Model file for the job. Use its own axes, mm. A direction names the side the tool comes from. Coordinates: 2 decimals unless noted, no trailing zeros. Write each loop counter-clockwise with the first axis right and the second up, starting at its lowest first coordinate (ties: lowest second). Pieces come first, ordered by that corner, then holes.
Q1. Band-saw the part on C-C, the plane z = 75.5. Write the cut outline in (x, y).
Q2. Which spindle directions (+Z, -Z, +X, -X, +Y, -Y) get a long thin tool onto all of the face, cutting with end or side? Do faces 1 (the flat face through (-16, -60, 16)), 2 (the flat face through (-20, -65, 54)), 3 (the flat face through (-1, -22, 32)), 4 (the flat face through (-54, -51, 20)), 5 (the flat face through (38, -51, 47)). Say none if no direction does.
Q3. Pull direction Y, two halves, no side cores. Call faces 6 (the flat face through (-29.126, -44.386, 54.477)), 7 (the flat face through (16, -60, 16)), 8 (the cylindrical face through (28.874, -66.959, 79.932)): released by +Y, released by -Y, zero draft, split by the parting line, or undercut.
Q4. Band-saw the part on B-B, the plane y = -15.5. Write the cut outline in (x, z), plus the area to 3 significant figures.
Q5. Pin check, flat tips, straight feed: P1, Ø16, axis at x = -4.5, z = 17, coming from the -Y side; P2, Ø3, axis at x = 29.5, y = 25, coming from the +Z side; P3, Ø5, axis at y = -61.5, z = 57.5, coming from the +X side; P4, Ø14.5, axis at y = -68, z = 72, coming from the -X side. Stop position of each tip, or through.
Q6. Band-saw the part on D-D, the plane x = 54. Write the cut outline in (y, z), plus the area to 3 significant figures.
Q7. Band-saw the part on A-A, the plane x = 0. Write the cut outline in (y, z).
Q8. Drill centre lines: probe 1 along Y at (x, z) = (-54, 8.5); probe 2 along X at (y, z) = (-65, 56); probe 3 along X at (y, z) = (-35.5, 15.5). Where is each one in solid material? Low to high.
from build123d import *

# Parameters (mm, degrees)
BASE_BLOCK_DEPTH              = 32
FORK_ARMS_DEPTH               = 20
SIDE_FLANGE_DEPTH             = 18
FLANGE_START                  = -18
FLANGE_EXTENSION_DEPTH        = 18
FORK_SLOT_SKETCH_W            = 32
FORK_SLOT_SKETCH_H            = 48
FORK_SLOT_48X32_DEPTH         = 123.849501423
FORK_ARM_PROFILE_CUT_SKETCH_R = 8
FORK_ARM_PROFILE_CUT_DEPTH    = 129.763348823
FLANGE_HOLES_SKETCH_R         = 8
FLANGE_HOLES_16_DEPTH         = 163.677595261
PIVOT_BORE_SKETCH_R           = 20
PIVOT_BORE_40_DEPTH           = 123.849501423


with BuildPart() as part:
    # Base Block Sketch → Base Block (new body)
    with BuildSketch(Plane.XY):
        with BuildLine():
            Line((-38, 0), (-38, -84))
            Line((-38, -84), (38, -84))
            Line((38, -84), (38, 0))
            ThreePointArc((38, 0), (0, 38), (-38, 0))
        make_face()
    extrude(amount=BASE_BLOCK_DEPTH)

    # Fork Arms Sketch → Fork Arms (add)
    with BuildSketch(Plane(origin=(0, 0, 0), x_dir=(-1, 0, 0), z_dir=(0, 0, -1))):
        with BuildLine():
            Line((38, -84), (70, -84))
            Line((70, -84), (70, -27.712812921))
            ThreePointArc((70, -27.712812921), (47.66969722, -21.166010489), (38, 0))
            Line((38, 0), (38, -84))
        make_face()
        with BuildLine():
            Line((-38, -84), (-70, -84))
            Line((-70, -84), (-70, -27.712812921))
            ThreePointArc((-70, -27.712812921), (-47.66969722, -21.166010489), (-38, 0))
            Line((-38, 0), (-38, -84))
        make_face()
    extrude(amount=-FORK_ARMS_DEPTH)

    # Side Flange Sketch → Side Flange (add)
    with BuildSketch(Plane.ZY.offset(38)):
        with BuildLine():
            Line((72, -84), (32, -84))
            Line((32, -84), (32, -36))
            Line((32, -36), (77.592604925, -53.009243843))
            ThreePointArc((77.592604925, -53.009243843), (87.745667634, -70.841469822), (72, -84))
        make_face()
    extrude(amount=-SIDE_FLANGE_DEPTH)

    # Flange Extension Sketch → Flange Extension (add)
    with BuildSketch(Plane(origin=(38, 0, 0), x_dir=(0, 0, -1), z_dir=(1, 0, 0)).offset(FLANGE_START)):
        with BuildLine():
            Line((-72, -84), (-32, -84))
            Line((-32, -84), (-32, -36))
            Line((-32, -36), (-77.592604925, -53.009243843))
            ThreePointArc((-77.592604925, -53.009243843), (-87.745667634, -70.841469822), (-72, -84))
        make_face()
    extrude(amount=FLANGE_EXTENSION_DEPTH)

    # Fork Slot Sketch → Fork Slot 48x32 (cut, through all)
    with BuildSketch(Plane.XY.offset(32)):
        with Locations((0, -60)):
            Rectangle(FORK_SLOT_SKETCH_W, FORK_SLOT_SKETCH_H)
    extrude(amount=-FORK_SLOT_48X32_DEPTH, mode=Mode.SUBTRACT)

    # Fork Arm Profile Cut Sketch → Fork Arm Profile Cut (cut, through all)
    with BuildSketch(Plane.XY.offset(20)):
        with Locations((-54, -41.856406461)):
            Circle(FORK_ARM_PROFILE_CUT_SKETCH_R)
        with Locations((-54, -69.856406461)):
            Circle(FORK_ARM_PROFILE_CUT_SKETCH_R)
        with Locations((54, -41.856406461)):
            Circle(FORK_ARM_PROFILE_CUT_SKETCH_R)
        with Locations((54, -69.856406461)):
            Circle(FORK_ARM_PROFILE_CUT_SKETCH_R)
    extrude(amount=-FORK_ARM_PROFILE_CUT_DEPTH, mode=Mode.SUBTRACT)

    # Flange Holes Sketch → Flange Holes _16 (cut, through all)
    with BuildSketch(Plane.ZY.offset(38)):
        with Locations(Location((72, -68, 0), (0, 0, 270))):
            Circle(FLANGE_HOLES_SKETCH_R)
    extrude(amount=-FLANGE_HOLES_16_DEPTH, mode=Mode.SUBTRACT)

    # Pivot Bore Sketch → Pivot Bore _40 (cut, through all)
    with BuildSketch(Plane.XY.offset(32)):
        Circle(PIVOT_BORE_SKETCH_R)
    extrude(amount=-PIVOT_BORE_40_DEPTH, mode=Mode.SUBTRACT)


solid = part.part
Answer sheet:
1. outline: (-38, -83.61) - (-20, -83.61) - (-20, -75.19) - (-38, -75.19) - close; (-38, -60.81) - (-20, -60.81) - (-20, -52.23) - (-38, -52.23) - close; (20, -83.61) - (38, -83.61) - (38, -75.19) - (20, -75.19) - close; (20, -60.81) - (38, -60.81) - (38, -52.23) - (20, -52.23) - close
2. face 1: +Z, -Z, -Y
2. face 2: +Z, +Y, -Y
2. face 3: +Z, +Y
2. face 4: +Z, -X, +Y, -Y
2. face 5: +Z, +X, +Y, -Y
3. face 6: released by +Y
3. face 7: zero draft
3. face 8: undercut
4. outline: (-42.68, 0) - (-12.64, 0) - (-12.64, 32) - (-38, 32) - (-38, 20) - (-42.68, 20) - close; (12.64, 0) - (42.68, 0) - (42.68, 20) - (38, 20) - (38, 32) - (12.64, 32) - close
4. area: 1,810 mm2
5. P1: stops at y = -36
5. P2: stops at z = 32
5. P3: stops at x = 38
5. P4: passes through
6. outline: (-84, 0) - (-77.86, 0) - (-77.86, 20) - (-84, 20) - close; (-61.86, 0) - (-49.86, 0) - (-49.86, 20) - (-61.86, 20) - close; (-33.86, 0) - (-25.3, 0) - (-25.3, 20) - (-33.86, 20) - close
6. area: 534 mm2
7. outline: (-36, 0) - (-20, 0) - (-20, 32) - (-36, 32) - close; (20, 0) - (38, 0) - (38, 32) - (20, 32) - close
8. probe 1: y = -84 to -77.86, -61.86 to -49.86, -33.86 to -25.3
8. probe 2: x = -38 to -20, 20 to 38
8. probe 3: x = -70 to -58.86, -49.14 to 49.14, 58.86 to 70
